Read the model definition and answer for the solid it produces. Units are mm, in the model's axes. Coordinates: 2 decimals unless noted, no trailing zeros. Write each loop counter-clockwise with the first axis right and the second up, starting at its lowest first coordinate (ties: lowest second). Pieces come first, ordered by that corner, then holes. Notation, with made-up numbers: M 60.25,75 L 107.25,75 A8 ccw 107.25,87 Z; hole C 75.25,53.25 d9. An arc over 180 degrees is marked long. Write item = value, one per line.
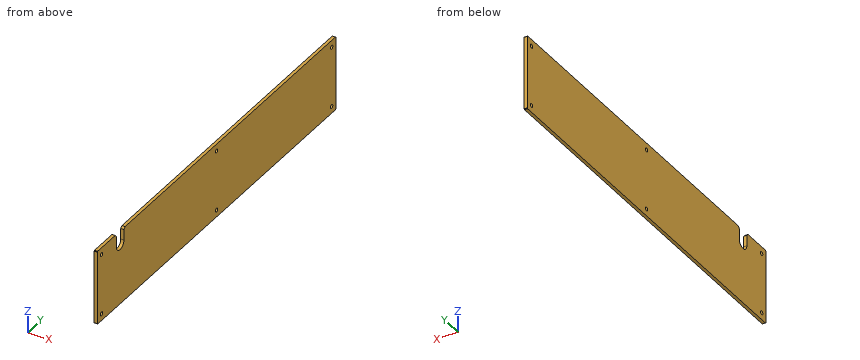
from build123d import *

# Parameters (mm, degrees)
SKETCH_1_W          = 118
SKETCH_1_H          = 628
EXTRUDE_1_DEPTH     = 5
CHAMFER_1_SIZE      = 1
SKETCH_2_R          = 3
CUT_EXTRUDE_1_DEPTH = 320.534035746
CUT_EXTRUDE_2_DEPTH = 320.534035746
CHAMFER_2_SIZE      = 3


with BuildPart() as part:
    # 草图1 → 凸台-拉伸1 (new body)
    with BuildSketch(Plane(origin=(0, 0, 0), x_dir=(0, 0, -1), z_dir=(1, 0, 0))):
        Rectangle(SKETCH_1_W, SKETCH_1_H)
    extrude(amount=EXTRUDE_1_DEPTH)

    # 倒角1
    chamfer_1_edges = [part.edges().sort_by_distance(p)[0] for p in [
        (2.5, 314, 59),
        (2.5, 314, -59),
        (2.5, -314, -59),
        (2.5, -314, 59),
    ]]
    chamfer(chamfer_1_edges, length=CHAMFER_1_SIZE)

    # 草图2 → 切除-拉伸1 (cut, through all)
    with BuildSketch(Plane.ZY):
        with Locations((-48, 303)):
            Circle(SKETCH_2_R)
        with Locations(Location((-48, -303, 0), (0, 0, 180))):
            Circle(SKETCH_2_R)
        with Locations((48, -303)):
            Circle(SKETCH_2_R)
        with Locations(Location((48, 303, 0), (0, 0, 180))):
            Circle(SKETCH_2_R)
        with Locations((48, 0)):
            Circle(SKETCH_2_R)
        with Locations((-48, 0)):
            Circle(SKETCH_2_R)
    extrude(amount=-CUT_EXTRUDE_1_DEPTH, mode=Mode.SUBTRACT)

    # 草图3 → 切除-拉伸2 (cut, through all)
    with BuildSketch(Plane(origin=(5, 0, 0), x_dir=(0, 0, -1), z_dir=(1, 0, 0))):
        with BuildLine():
            Line((-39, -264), (-59, -264))
            ThreePointArc((-59, -264), (-69, -254), (-59, -244))
            Line((-59, -244), (-39, -244))
            ThreePointArc((-39, -244), (-29, -254), (-39, -264))
        make_face()
    extrude(amount=-CUT_EXTRUDE_2_DEPTH, mode=Mode.SUBTRACT)

    # 倒角2
    chamfer_2_edges = [part.edges().sort_by_distance(p)[0] for p in [
        (2.5, -264, 59),
        (2.5, -244, 59),
    ]]
    chamfer(chamfer_2_edges, length=CHAMFER_2_SIZE)


solid = part.part
Item 1: A flat-ended cylindrical pin translates along its axis: pin 1 (12 mm diameter, centred on y = 128.5, z = -8, fed in from -X). Find the tip coordinate at first contact, or state that the pin passes through.
Worked answers:
pin_1 = 0
Item 2: Consider line 1 along Y through (x, z) = (2.4, 48); line 2 along Y through (x, z) = (1.35, -48); line 3 along Z through (x, y) = (2.2, -303). Determine where each line is inside the solid, lowest interval first. Write a range as from..to.
Worked answers:
line_1 = -314..-306, -300..-264, -244..-3, 3..300, 306..314
line_2 = -314..-306, -300..-3, 3..300, 306..314
line_3 = -59..-51, -45..45, 51..59
Item 3: Find section A-A (y = -254). Determine the outline of the cut face in (x, z), and give its area (3 significant figures).
Worked answers:
outline = M 0,-59 L 5,-59 L 5,29 L 0,29 Z
area = 440 mm²
